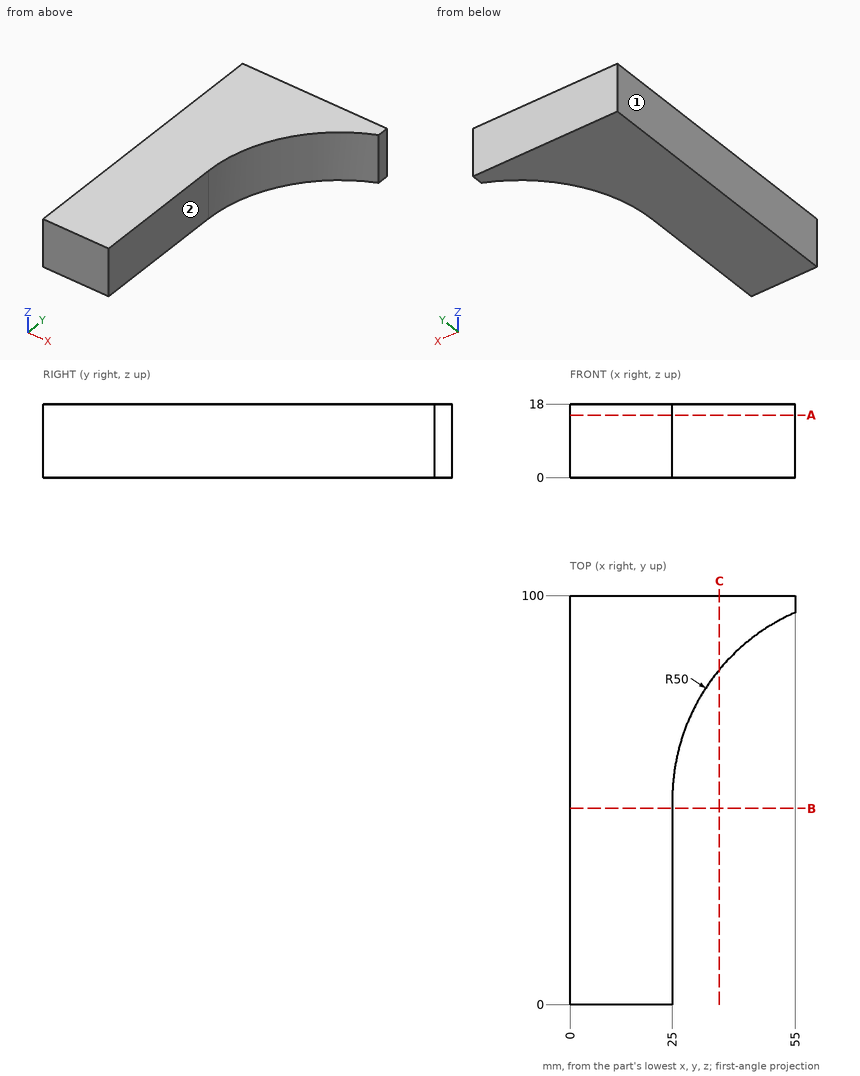
For this review, use the dimensioned drawing (mm, ordinates from the lowest corner) and the shaded views. A direction names the side the tool comes from. Give positions to 0.01 mm unless a question says otherwise; leave off trailing zeros. Order: outer loops, then holes, each group sorted by start corner. A loop starts at its lowest first (then second) coordinate and runs counter-clockwise, first axis right, second up. Notation, with made-up numbers: M 44,-2 L 66,-2 A30 ccw 66,30 Z; hole C 23,-25 d10. An arc over 180 degrees is marked long. One line per question, with ' | ' between items. Start each with the question number.
1) For the marked faces 1 and 2, list the 3-axis set-ups (+Z, -Z, +X, -X, +Y, -Y) from which the entire face can be reached by the end or side of a thin tool; tool diameter is ignored.
2) Wall thickness on L1, parallel to X at y = 17, z = 6.5; L2, parallel to X at y = 67, z = 16.5; L3, parallel to Y at x = 31, z = 8: over which ranges is each line inside the solid? List them lowest first. Write a range as from..to.
3) Clearance check with flat-ended pins moving along their axes: P1, Ø4, axis at y = 66, z = 5, coming from the +X side; P2, Ø4, axis at x = 43, z = 10.5, coming from the -Y side. State where each tip first meets the part, or that it passes through.
4) Consider section B-B, the plane y = 48. Give the boundary of the cut face in (x, z).
5) Consider section A-A, the plane z = 15.25. Give the boundary of the cut face in (x, y), then the cut area to 3 significant figures.
6) Consider section C-C, the plane x = 36.5. Give the boundary of the cut face in (y, z), then the cut area to 3 significant figures.
Found:
1) face 1: +Z, -Z, -X, +Y, -Y | face 2: +Z, -Z, +X, -Y
2) L1: x = 0..25 | L2: x = 0..27.98 | L3: y = 73.75..100
3) P1: stops at x = 28.35 | P2: stops at y = 86.66
4) outline: M 0,0 L 25,0 L 25,18 L 0,18 Z
5) outline: M 0,0 L 25,0 L 25,50 A50 cw 55,95.83 L 55,100 L 0,100 Z | area: 3,010 mm²
6) outline: M 81.9,0 L 100,0 L 100,18 L 81.9,18 Z | area: 326 mm²
